Geometry check sheet. Reference: drawing and pictorial views, mm from the part's lowest x, y, z. Give positions to 0.01 mm unless a question says otherwise; leave off trailing zeros. Write each loop counter-clockwise with the first axis right and the second up, starting at its lowest first coordinate (ties: lowest second). Pieces come first, ordered by that corner, then holes.
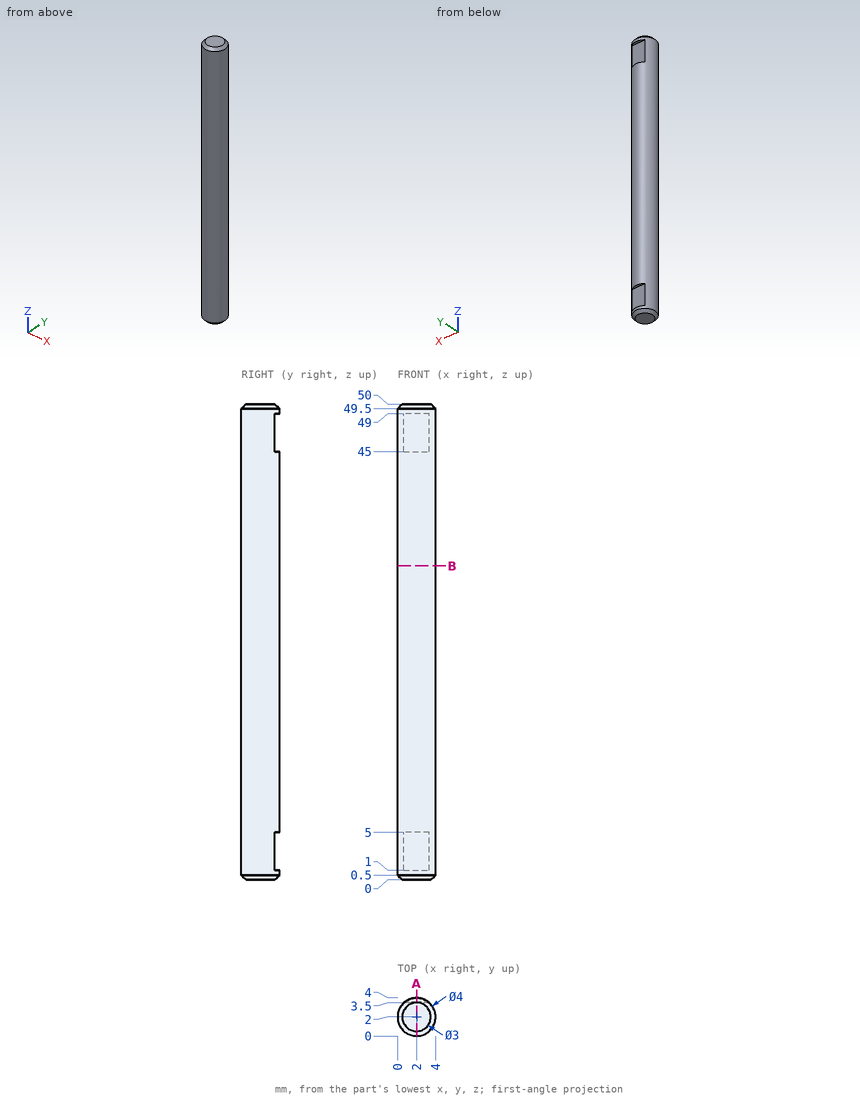
Item 1: Sectioned sample at B-B on z = 33. Record the cut outline in (x, y).
Answer key:
outline: circle Ø4 at (2, 2)
Item 2: Scan lines: line 1 along Z through (x, y) = (1.7, 3.65); line 2 along Y through (x, z) = (2.15, 7.5); line 3 along X through (y, z) = (2.1, 9). Record each from-to range of solid material in increasing order.
Answer key:
line 1: z = 0.18 to 1, 5 to 45, 49 to 49.82
line 2: y = 0.01 to 3.99
line 3: x = 0 to 4
Item 3: Depth check by flat-ended pin: pin 1 (0.6 mm diameter, centred on x = 1.5, y = 4, fed in from -Z); pin 2 (0.8 mm diameter, centred on x = 1.5, z = 46.5, fed in from +Y). Enter the tip coordinate at first touch or a pass-through.
Answer key:
pin 1: stops at z = 0.26
pin 2: stops at y = 3.5
Item 4: Sectioned sample at A-A on x = 2. Record the cut outline in (y, z), then the cut area to 4 significant figures.
Answer key:
outline: (0, 0.5) - (0.5, 0) - (3.5, 0) - (4, 0.5) - (4, 1) - (3.5, 1) - (3.5, 5) - (4, 5) - (4, 45) - (3.5, 45) - (3.5, 49) - (4, 49) - (4, 49.5) - (3.5, 50) - (0.5, 50) - (0, 49.5) - close
area: 195.5 mm2
